from build123d import *

# Parameters (mm, degrees)
SKETCH_1_3_W          = 40.6
SKETCH_1_3_H          = 60
BOSS_EXTRUDE1_DEPTH   = 15.3
SKETCH_1_3_2_W        = 19.4
SKETCH_1_3_2_H        = 60
BOSS_EXTRUDE2_DEPTH   = 7.3
SKETCH2_W             = 40.6
SKETCH2_H             = 9
BOSS_EXTRUDE3_DEPTH   = 7
M3_TAPPED_HOLE1_D     = 2.5
M3_TAPPED_HOLE1_DEPTH = 7.5
M3_TAPPED_HOLE1_TIP   = 0.751075774
M3_TAPPED_HOLE2_D     = 2.5
M3_TAPPED_HOLE2_DEPTH = 7.5
M3_TAPPED_HOLE2_TIP   = 0.751075774
FILLET1_R             = 5
SKETCH11_W            = 42
SKETCH11_H            = 4.723838164
CUT_EXTRUDE5_DEPTH    = 73.78462902
SKETCH12_R            = 3.75
CUT_EXTRUDE6_DEPTH    = 19.3
SKETCH13_R            = 2.2
CUT_EXTRUDE7_DEPTH    = 52.321618612


with BuildPart() as part:
    # Sketch 1_3 → Boss-Extrude1 (new body)
    with BuildSketch(Plane(origin=(0, 0, 0), x_dir=(1, 0, 0), z_dir=(0, 1, 0))):
        with Locations((7.125373134, -4.645522388)):
            Rectangle(SKETCH_1_3_W, SKETCH_1_3_H)
    extrude(amount=BOSS_EXTRUDE1_DEPTH)

    # Sketch 1_3 2 → Boss-Extrude2 (add)
    with BuildSketch(Plane(origin=(0, 0, 0), x_dir=(1, 0, 0), z_dir=(0, 1, 0))):
        with Locations((-22.874626866, -4.645522388)):
            Rectangle(SKETCH_1_3_2_W, SKETCH_1_3_2_H)
    extrude(amount=BOSS_EXTRUDE2_DEPTH)

    # Sketch2 → Boss-Extrude3 (add)
    with BuildSketch(Plane(origin=(0, 15.3, 0), x_dir=(1, 0, 0), z_dir=(0, 1, 0))):
        with Locations((7.125373134, -30.145522388)):
            Rectangle(SKETCH2_W, SKETCH2_H)
    extrude(amount=BOSS_EXTRUDE3_DEPTH)

    # M3 Tapped Hole1
    with Locations(Plane(origin=(0, 7.3, 0), x_dir=(1, 0, 0), z_dir=(0, 1, 0))):
        with Locations((-27.574626866, -2.445522388), (-27.574626866, -26.445522388)):
            Hole(M3_TAPPED_HOLE1_D / 2, depth=M3_TAPPED_HOLE1_DEPTH)
            with Locations((0, 0, -(M3_TAPPED_HOLE1_DEPTH + M3_TAPPED_HOLE1_TIP / 2))):  # 118° drill point
                Cone(0, M3_TAPPED_HOLE1_D / 2, M3_TAPPED_HOLE1_TIP, mode=Mode.SUBTRACT)

    # M3 Tapped Hole2
    with Locations(Plane(origin=(0, 15.3, 0), x_dir=(1, 0, 0), z_dir=(0, 1, 0))):
        with Locations((-10.174626866, -14.945522388), (17.825373134, -14.945522388), (-2.674626866, 17.534477612), (10.325373134, 17.534477612)):
            Hole(M3_TAPPED_HOLE2_D / 2, depth=M3_TAPPED_HOLE2_DEPTH)
            with Locations((0, 0, -(M3_TAPPED_HOLE2_DEPTH + M3_TAPPED_HOLE2_TIP / 2))):  # 118° drill point
                Cone(0, M3_TAPPED_HOLE2_D / 2, M3_TAPPED_HOLE2_TIP, mode=Mode.SUBTRACT)

    # Fillet1
    fillet1_edges = [part.edges().sort_by_distance(p)[0] for p in [
        (-32.574626866, 3.65, -25.354477612),
        (-32.574626866, 3.65, 34.645522388),
        (27.425373134, 11.15, 34.645522388),
        (27.425373134, 7.65, -25.354477612),
    ]]
    fillet(fillet1_edges, radius=FILLET1_R)

    # Sketch11 → Cut-Extrude5 (cut, through all)
    with BuildSketch(Plane.ZY.offset(32.574626866)):
        with Locations((4.645522388, -1.861919082)):
            Rectangle(SKETCH11_W, SKETCH11_H)
    extrude(amount=-CUT_EXTRUDE5_DEPTH, mode=Mode.SUBTRACT)

    # Sketch12 → Cut-Extrude6 (cut)
    with BuildSketch(Plane(origin=(0, 22.3, 0), x_dir=(1, 0, 0), z_dir=(0, 1, 0))):
        with Locations(Location((21.425373134, 19.354477612, 0), (0, 0, 270))):
            Circle(SKETCH12_R)
        with Locations(Location((-26.574626866, 19.354477612, 0), (0, 0, 270))):
            Circle(SKETCH12_R)
        with Locations(Location((-2.574626866, -29.895522388, 0), (0, 0, 270))):
            Circle(SKETCH12_R)
    extrude(amount=-CUT_EXTRUDE6_DEPTH, mode=Mode.SUBTRACT)

    # Sketch13 → Cut-Extrude7 (cut, through all)
    with BuildSketch(Plane(origin=(0, 3, 0), x_dir=(1, 0, 0), z_dir=(0, 1, 0))):
        with Locations(Location((-2.574626866, -29.895522388, 0), (0, 0, 270))):
            Circle(SKETCH13_R)
        with Locations(Location((21.425373134, 19.354477612, 0), (0, 0, 270))):
            Circle(SKETCH13_R)
        with Locations(Location((-26.574626866, 19.354477612, 0), (0, 0, 270))):
            Circle(SKETCH13_R)
    extrude(amount=-CUT_EXTRUDE7_DEPTH, mode=Mode.SUBTRACT)


solid = part.part
For this review, take the finished solid that the model builds, in its own axes (mm). A direction names the side the tool comes from. Round coordinates to 2 decimals unless told otherwise and drop trailing zeros. Order: outer loops, then holes, each group sorted by start corner. A loop starts at its lowest first (then second) coordinate and runs counter-clockwise, first axis right, second up. Notation, with made-up numbers: (46, 54) -> (61, 54) arc R9 ccw to (61, 58) -> close; hole circle Ø2 at (-33, -8). An arc over 180 degrees is marked (long way). Write item = value, one per line. Start each with the question number.
1) To check wall thickness, follow line 1 (X direction, y = 2.75, z = 30); line 2 (Z direction, x = 14.5, y = 18.75); line 3 (X direction, y = 12.25, z = -0.5). State the ranges of each line that lie inside material, in increasing order. Write a range as from..to.
2) Tool access review of faces 5 (the face through (-3, 0.5, 4)), 6 (the face through (19, 3, -19)), 7 (the face through (-3, 0, 33)), 8 (the face through (-13.175, 11, 5)), 9 (the face through (23.3, 1.5, -18.2)): name each direction out of +Z, -Z, +X, -X, +Y, -Y from which nothing blocks a thin tool from reaching the whole face with its end or side.
3) The part is to be moulded in two halves that separate along Z. For faces 1 (the face through (-31.07, 3.7, 33.22)), 2 (the face through (19.074, 11.498, 14.891)), 3 (the face through (-10.2, 7.18, 14.73)), 4 (the face through (7, 22.3, 30)), say which applies: +Z half, -Z half, draft (parallel to the pull), parting line (faces both ways), or undercut.
4) Take a section at C-C on y = 18.25. State the section outline as (x, z) points.
5) Insertion check: pin 1 (8 mm diameter, centred on x = 11, z = 19.5, fed in from -Y); pin 2 (2.5 mm diameter, centred on x = -26.57, z = -19.35, fed in from +Y); pin 3 (7.5 mm diameter, centred on y = 11.5, z = 11, fed in from -X); pin 4 (5.5 mm diameter, centred on x = 1.5, y = 18.5, fed in from -Z). Each pin has a flat end and moves straight along its axis. Give the tip position at first contact, or say it passes through.
6) Take a section at A-A on x = -19. State the section outline as (y, z) points, plus the area to 3 significant figures.
7) Take a section at B-B on z = 4.5. State the section outline as (x, y) points.
8) Take a section at D-D on x = 15. State the section outline as (y, z) points, plus the area to 3 significant figures.
Verdict:
q1.line_1 = -32.56..-4.77, -0.38..27.41
q1.line_2 = 25.65..34.65
q1.line_3 = -13.17..27.43
q2.face_5 = +X, -X, -Y
q2.face_6 = +Y
q2.face_7 = +Z, -Z, +X, -X, -Y
q2.face_8 = +Z, -Z, -X, +Y
q2.face_9 = +Y, -Y
q3.face_1 = +Z half
q3.face_2 = undercut
q3.face_3 = undercut
q3.face_4 = draft
q4.outline = (-13.17, 25.65) -> (27.43, 25.65) -> (27.43, 29.65) arc R5 ccw to (22.43, 34.65) -> (-13.17, 34.65) -> close; hole circle Ø7.5 at (-2.57, 29.9)
q5.pin_1 = 0.5
q5.pin_2 = through
q5.pin_3 = -13.17
q5.pin_4 = 25.65
q6.outline = (0, -25.35) -> (7.3, -25.35) -> (7.3, 34.65) -> (0, 34.65) -> (0, 25.65) -> (0.5, 25.65) -> (0.5, -16.35) -> (0, -16.35) -> close
q6.area = 417 mm2
q7.outline = (-32.57, 0.5) -> (27.43, 0.5) -> (27.43, 15.3) -> (-13.17, 15.3) -> (-13.17, 7.3) -> (-32.57, 7.3) -> close
q8.outline = (0, -25.35) -> (15.3, -25.35) -> (15.3, 25.65) -> (22.3, 25.65) -> (22.3, 34.65) -> (0, 34.65) -> (0, 25.65) -> (0.5, 25.65) -> (0.5, -16.35) -> (0, -16.35) -> close
q8.area = 960 mm2
